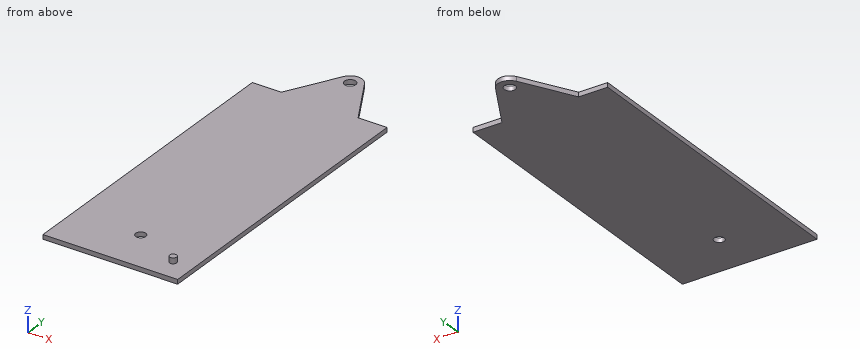
```python
from build123d import *

# Parameters (mm, degrees)
SKETCH1_R           = 10
SKETCH1_R_2         = 9
BOSS_EXTRUDE1_DEPTH = 8
SKETCH2_R           = 6
BOSS_EXTRUDE2_DEPTH = 10


with BuildPart() as part:
    # Sketch1 → Boss-Extrude1 (new body)
    with BuildSketch(Plane.XY):
        with BuildLine():
            Line((-120, 550), (-68.4, 550))
            Line((-68.4, 550), (-18.684224353, 640.288176603))
            ThreePointArc((-18.684224353, 640.288176603), (0, 651.329482354), (18.684224353, 640.288176603))
            Line((18.684224353, 640.288176603), (68.4, 550))
            Line((68.4, 550), (120, 550))
            Line((120, 550), (120, 0))
            Line((120, 0), (-120, 0))
            Line((-120, 0), (-120, 550))
        make_face()
        with Locations((0, 630)):
            Circle(SKETCH1_R, mode=Mode.SUBTRACT)
        with Locations((0, 80)):
            Circle(SKETCH1_R_2, mode=Mode.SUBTRACT)
    extrude(amount=BOSS_EXTRUDE1_DEPTH)

    # Sketch2 → Boss-Extrude2 (add)
    with BuildSketch(Plane.XY.offset(8)):
        with Locations((85, 40)):
            Circle(SKETCH2_R)
    extrude(amount=BOSS_EXTRUDE2_DEPTH)


solid = part.part
```
Model file for the job. Use its own axes, mm. Give positions to 0.01 mm unless a question says otherwise; leave off trailing zeros. Write each loop counter-clockwise with the first axis right and the second up, starting at its lowest first coordinate (ties: lowest second). Pieces come first, ordered by that corner, then holes. Notation, with made-up numbers: (41, -1) - (84, -1) arc R28 cw to (84, 32) - close; hole circle Ø6 at (-31, 59). An arc over 180 degrees is marked (long way). One line per question, with ' | ' between items. Start each with the question number.
(1) Slice it at D-D on y = 40. Write the cut outline in (x, z).
(2) Wall check: line 1 along Y through (x, z) = (0, 2); line 2 along Z through (x, y) = (-28, 411.5); line 3 along X through (y, z) = (630, 1.5). Give the ranges that are in metal, low to high. Write a range as from..to.
(3) Slice it at B-B on y = 630. Write the cut outline in (x, z).
(4) Pin check, flat tips, straight feed: P1, Ø10, axis at x = -43.5, z = 14.5, coming from the +Y side; P2, Ø2, axis at x = -41, z = 2.5, coming from the +Y side; P3, Ø6.5, axis at x = 100.5, z = 2.5, coming from the +Y side. Stop position of each tip, or through.
(5) Slice it at C-C on z = 2.75. Write the cut outline in (x, y).
(6) Slice it at A-A on x = 0. Write the cut outline in (y, z), plus the area to 3 significant figures.
Results below:
1) outline: (-120, 0) - (120, 0) - (120, 8) - (91, 8) - (91, 18) - (79, 18) - (79, 8) - (-120, 8) - close
2) line 1: 0..71, 89..620, 640..651.33 | line 2: 0..8 | line 3: -24.35..-10, 10..24.35
3) outline: (-24.35, 0) - (-10, 0) - (-10, 8) - (-24.35, 8) - close; (10, 0) - (24.35, 0) - (24.35, 8) - (10, 8) - close
4) P1: through | P2: y = 601.58 | P3: y = 550
5) outline: (-120, 0) - (120, 0) - (120, 550) - (68.4, 550) - (18.68, 640.29) arc R21.33 ccw to (-18.68, 640.29) - (-68.4, 550) - (-120, 550) - close; hole circle Ø20 at (0, 630); hole circle Ø18 at (0, 80)
6) outline: (0, 0) - (71, 0) - (71, 8) - (0, 8) - close; (89, 0) - (620, 0) - (620, 8) - (89, 8) - close; (640, 0) - (651.33, 0) - (651.33, 8) - (640, 8) - close | area: 4,910 mm^2
